Can you work these out from the model? Positions are in its coordinate system, mm. Face numbers are marked on the shaded views. A direction names the side the tool comes from. Round coordinates to 2 decimals unless told otherwise and drop trailing zeros. Loops run counter-clockwise (first coordinate to the right, second up) from the corner with the lowest first, then second, coordinate; pieces in that order, holes last.
(1) Thinking about a two-plate mould opening in Z: for the marked faces 3, 4 and 5, which applies, released by +Z, released by -Z, zero draft, split by the parting line, or undercut?
(2) If I drill on line 1 along Z through (x, y) = (0.25, -34.5); line 2 along Z through (x, y) = (-5.75, -6.5); line 3 along Y through (x, z) = (0, -210), over which ranges is the centre line in solid material (lowest first)?
(3) Which directions (+Z, -Z, +X, -X, +Y, -Y) give clear straight access to the entire face, cutting with the end or side of a thin tool? Please do the marked faces 1 and 2.
(4) I want a section at A-A on y = 0. Write out the boundary of the cut face in (x, z).
(5) I want a section at D-D on y = -50. Write out the boundary of the cut face in (x, z), plus the area to 3 significant figures.
(6) I want a section at C-C on z = -39. Write out the boundary of the cut face in (x, y), plus the area to 3 significant figures.
(7) I want a section at B-B on x = 0. Write out the boundary of the cut face in (y, z), plus the area to 3 significant figures.
(8) Will these pins go through, and if not, where does the flat tip stop? pin 1 Ø1 at (x, z) = (3, -69) entering from +Y; pin 2 Ø1 at (x, y) = (2, -14.5) entering from +Z; pin 3 Ø2 at (x, y) = (1.5, -36.5) entering from -Z.
from build123d import *

# Parameters (mm, degrees)
SKETCH_1_R = 7


with BuildPart() as part:
    # 扫描1: sweep along a path in 草图3
    with BuildLine(Plane(origin=(0, 0, 0), x_dir=(0, 0, -1), z_dir=(1, 0, 0))) as sweep_1_path:
        Line((0, 0), (80, 0))
        Line((80, 0), (80, -50))
        Line((80, -50), (160, -50))
        Line((160, -50), (160, 0))
        Line((160, 0), (220, 0))
    # 草图1 → 扫描1 (sweep)
    with BuildSketch(Plane.XY):
        Circle(SKETCH_1_R)
    sweep(path=sweep_1_path.line, transition=Transition.RIGHT)


solid = part.part
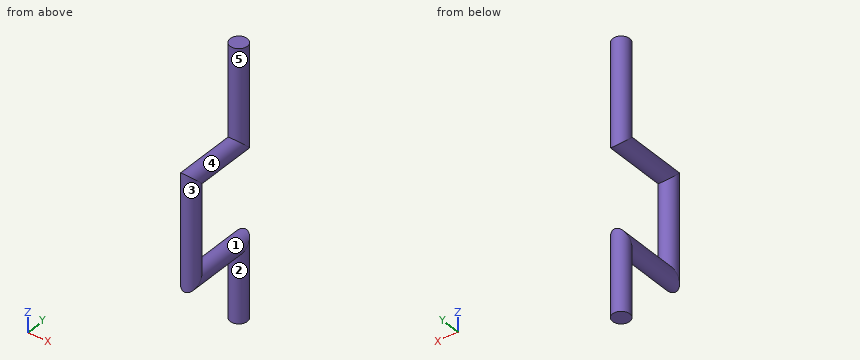
Filled sheet:
1. face 3: undercut
1. face 4: undercut
1. face 5: zero draft
2. line 1: z = -167 to -153, -87 to -73
2. line 2: z = -163.99 to -156.01, -83.99 to -76.01
2. line 3: y = -7 to 7
3. face 1: none
3. face 2: -Z
4. outline: (-7, -220) - (7, -220) - (7, -160) arc R7 ccw to (-7, -160) - close; (-7, -80) arc R7 ccw to (7, -80) - (7, 0) - (-7, 0) - close
5. outline: (-7, -160) arc R7 ccw to (7, -160) - (7, -80) arc R7 ccw to (-7, -80) - close
5. area: 1,270 mm2
6. outline: circle Ø14 at (0, 0)
6. area: 154 mm2
7. outline: (-57, -167) - (-7, -167) - (-7, -220) - (7, -220) - (7, -153) - (-43, -153) - (-43, -87) - (7, -87) - (7, 0) - (-7, 0) - (-7, -73) - (-57, -73) - close
7. area: 4,480 mm2
8. pin 1: stops at y = 6.54
8. pin 2: stops at z = -73.16
8. pin 3: stops at z = -166.98
